Can you work these out from the model? Positions are in its coordinate system, mm. A direction names the side the tool comes from. Give positions to 0.01 mm unless a question says otherwise; leave off trailing zeros. Loops run counter-clockwise (first coordinate to the right, second up) from the corner with the lowest first, then second, coordinate; pieces in that order, holes last. Notation, with made-up numbers: (41.5, 60) - (85.5, 60) arc R15 ccw to (85.5, 71) - close; hole circle Ø2 at (35.5, -35.75). An arc over 180 degrees is marked (long way). Answer in a Markdown table with one row per item.
from build123d import *

# Parameters (mm, degrees)
SKETCH_1_W                   = 65
SKETCH_1_H                   = 50
EXTRUDE_1_DEPTH              = 9
SKETCH_4_W                   = 2
SKETCH_4_H                   = 34
CUT_EXTRUDE_1_DEPTH          = 71.221079456
HOLE_WIZARD_M4_1_D           = 4.5
HOLE_WIZARD_M4_1_CBORE_D     = 8
HOLE_WIZARD_M4_1_CBORE_DEPTH = 4.4
SKETCH_8_W                   = 15
SKETCH_8_H                   = 50
CUT_EXTRUDE_3_DEPTH          = 2
F_6_0MM_1_D                  = 6
F_6_0MM_1_DEPTH              = 7
F_6_0MM_1_TIP                = 1.802581857
HOLE_WIZARD_M6_2_D           = 6.6
HOLE_WIZARD_M6_2_CBORE_D     = 11
HOLE_WIZARD_M6_2_CBORE_DEPTH = 9
HOLE_WIZARD_M6_1_D           = 5
HOLE_WIZARD_M6_1_DEPTH       = 15
HOLE_WIZARD_M6_1_TIP         = 1.502151548
F_6_0MM_2_D                  = 6
F_6_0MM_2_DEPTH              = 6
F_6_0MM_2_TIP                = 1.802581857


with BuildPart() as part:
    # 草图1 → 凸台-拉伸1 (new, symmetric)
    with BuildSketch(Plane.XY):
        Rectangle(SKETCH_1_W, SKETCH_1_H)
    extrude(amount=EXTRUDE_1_DEPTH, both=True)

    # 草图4 → 切除-拉伸1 (cut, through all)
    with BuildSketch(Plane(origin=(32.5, 0, 0), x_dir=(0, 0, -1), z_dir=(1, 0, 0))):
        with Locations((8, 0)):
            Rectangle(SKETCH_4_W, SKETCH_4_H)
    extrude(amount=-CUT_EXTRUDE_1_DEPTH, mode=Mode.SUBTRACT)

    # Hole Wizard M4 _1 (through all)
    with Locations(Plane.XY.offset(9)):
        with Locations((11.2, -13), (-14.8, -13), (-14.8, 13), (11.2, 13)):
            CounterBoreHole(HOLE_WIZARD_M4_1_D / 2, HOLE_WIZARD_M4_1_CBORE_D / 2, HOLE_WIZARD_M4_1_CBORE_DEPTH)

    # 草图8 → 切除-拉伸3 (cut)
    with BuildSketch(Plane.XY.offset(9)):
        with Locations((-1.8, 0)):
            Rectangle(SKETCH_8_W, SKETCH_8_H)
    extrude(amount=-CUT_EXTRUDE_3_DEPTH, mode=Mode.SUBTRACT)

    # Ø6.0mm 暗销孔1
    with Locations(Plane.XY.offset(7)):
        with Locations((-1.8, 0)):
            Hole(F_6_0MM_1_D / 2, depth=F_6_0MM_1_DEPTH)
            with Locations((0, 0, -(F_6_0MM_1_DEPTH + F_6_0MM_1_TIP / 2))):  # 118° drill point
                Cone(0, F_6_0MM_1_D / 2, F_6_0MM_1_TIP, mode=Mode.SUBTRACT)

    # M6 六角凹头螺钉的柱形沉头孔2 (through all)
    with Locations(Plane(origin=(0, 0, -9), x_dir=(-1, 0, 0), z_dir=(0, 0, -1))):
        with Locations((1.8, 17.5), (1.8, -17.5)):
            CounterBoreHole(HOLE_WIZARD_M6_2_D / 2, HOLE_WIZARD_M6_2_CBORE_D / 2, HOLE_WIZARD_M6_2_CBORE_DEPTH)

    # M6 螺纹孔1
    with Locations(Plane(origin=(0, 25, 0), x_dir=(1, 0, 0), z_dir=(0, 1, 0))):
        with Locations((20.5, 0), (-26.5, 0)):
            Hole(HOLE_WIZARD_M6_1_D / 2, depth=HOLE_WIZARD_M6_1_DEPTH)
            with Locations((0, 0, -(HOLE_WIZARD_M6_1_DEPTH + HOLE_WIZARD_M6_1_TIP / 2))):  # 118° drill point
                Cone(0, HOLE_WIZARD_M6_1_D / 2, HOLE_WIZARD_M6_1_TIP, mode=Mode.SUBTRACT)

    # Ø6.0mm 暗销孔2
    with Locations(Plane(origin=(0, 25, 0), x_dir=(1, 0, 0), z_dir=(0, 1, 0))):
        with Locations((7, 0), (-13, 0)):
            Hole(F_6_0MM_2_D / 2, depth=F_6_0MM_2_DEPTH)
            with Locations((0, 0, -(F_6_0MM_2_DEPTH + F_6_0MM_2_TIP / 2))):  # 118° drill point
                Cone(0, F_6_0MM_2_D / 2, F_6_0MM_2_TIP, mode=Mode.SUBTRACT)


solid = part.part
Q1. On a 3-axis mill with a long thin cutter (end or side, diameter ignored), from which of +Z, -Z, +X, -X, +Y, -Y can I reach the whole of each face in a straight line? I mean faces 4 (the face through (-2, 14, 0)), 5 (the face through (-10, 22, 0)), 6 (the face through (-9.3, 0, 8)). Say none if no direction works.
Checked values:
| item | result |
|---|---|
| face 4 | -Z |
| face 5 | +Y |
| face 6 | +Z, +Y, -Y |
Q2. Imagine slicing it at D-D, the plane x = -22.5. Write out the boundary of the cut face in (y, z).
Checked values:
| item | result |
|---|---|
| outline | (-25, -9) - (-17, -9) - (-17, -7) - (17, -7) - (17, -9) - (25, -9) - (25, 9) - (-25, 9) - close |
Q3. If I drill on line 1 (Y direction, x = 11.2, z = -4); line 2 (Y direction, x = -16, z = 7.75); line 3 (Z direction, x = -16, y = -16), over which ranges is the centre line in solid material (lowest first)? Write a range as [from, to].
Checked values:
| item | result |
|---|---|
| line 1 | y = [-25, -15.25], [-10.75, 10.75], [15.25, 25] |
| line 2 | y = [-25, -16.82], [-9.18, 9.18], [16.82, 25] |
| line 3 | z = [-7, 4.6] |
Q4. If we mould it in two halves opening along Y, with no side actions, what happens to faces 1 (the face through (0, 25, 0)), 2 (the face through (-24, 17, 0)), 3 (the face through (18, 17, -8))? For each: released by +Y, released by -Y, zero draft, split by the parting line, or undercut.
Checked values:
| item | result |
|---|---|
| face 1 | released by +Y |
| face 2 | zero draft |
| face 3 | undercut |
Q5. Imagine slicing it at B-B, the plane y = -7. Write out the boundary of the cut face in (x, z).
Checked values:
| item | result |
|---|---|
| outline | (-32.5, -7) - (32.5, -7) - (32.5, 9) - (5.7, 9) - (5.7, 7) - (-9.3, 7) - (-9.3, 9) - (-32.5, 9) - close |
Q6. For pin 1 (3.5 mm diameter, centred on x = 7, z = 0, fed in from +Y); pin 2 (5 mm diameter, centred on x = 11.2, y = 13, fed in from -Z); pin 3 (7 mm diameter, centred on x = 11.2, y = -13, fed in from +Z), each with a flat end and sliding along its axis, tell me the tip position at first contact or that it passes through.
Checked values:
| item | result |
|---|---|
| pin 1 | stops at y = 18.25 |
| pin 2 | stops at z = -7 |
| pin 3 | stops at z = 4.6 |
Q7. Imagine slicing it at C-C, the plane z = 6. Write out the boundary of the cut face in (x, y).
Checked values:
| item | result |
|---|---|
| outline | (-32.5, -25) - (32.5, -25) - (32.5, 25) - (-32.5, 25) - close; hole circle Ø8 at (-14.8, -13); hole circle Ø8 at (-14.8, 13); hole circle Ø6.6 at (-1.8, -17.5); hole circle Ø6.6 at (-1.8, 17.5); hole circle Ø6 at (-1.8, 0); hole circle Ø8 at (11.2, -13); hole circle Ø8 at (11.2, 13) |
Q8. Imagine slicing it at A-A, the plane x = 11.2. Write out the boundary of the cut face in (y, z), and give its area (3 significant figures).
Checked values:
| item | result |
|---|---|
| outline | (-25, -9) - (-17, -9) - (-17, -7) - (-15.25, -7) - (-15.25, 4.6) - (-17, 4.6) - (-17, 9) - (-25, 9) - close; (-10.75, -7) - (10.75, -7) - (10.75, 4.6) - (9, 4.6) - (9, 9) - (-9, 9) - (-9, 4.6) - (-10.75, 4.6) - close; (15.25, -7) - (17, -7) - (17, -9) - (25, -9) - (25, 9) - (17, 9) - (17, 4.6) - (15.25, 4.6) - close |
| area | 657 mm² |
